Build history of the part. All positions in model axes, mm. A direction names the side the tool comes from. Coordinates: 2 decimals unless noted, no trailing zeros. Write each loop counter-clockwise with the first axis right and the second up, starting at its lowest first coordinate (ties: lowest second). Pieces come first, ordered by that corner, then holes.
from build123d import *

# Parameters (mm, degrees)
BASE_DISC_SKETCH_R           = 90
BASE_DISC_180_DEPTH          = 15
CLAMP_FRAME_WALL_DEPTH       = 70
TOP_JAW_PLATE_DEPTH          = 15
TABLE_RISER_SKETCH_R         = 60
TABLE_RISER_SKETCH_R_2       = 40
TABLE_RISER_DEPTH            = 40
RISER_START                  = -30
RISER_SLOTS_CUT_DEPTH        = 30
TABLE_PLATE_SKETCH_R         = 60
TABLE_PLATE_120_DEPTH        = 5
TABLE_BOLT_HOLES_SKETCH_R    = 5
TABLE_BOLT_HOLES_4X_10_DEPTH = 20
TABLE_RING_SKETCH_R          = 40
TABLE_RING_SKETCH_R_2        = 30
TABLE_RING_80_DEPTH          = 15
CENTRE_SPIGOT_SKETCH_R       = 20
CENTRE_SPIGOT_40_DEPTH       = 25


with BuildPart() as part:
    # Base Disc Sketch → Base Disc _180 (new body)
    with BuildSketch(Plane(origin=(0, 0, 0), x_dir=(1, 0, 0), z_dir=(0, 1, 0))):
        with Locations(Location((0, 0, 0), (0, 0, 270))):
            Circle(BASE_DISC_SKETCH_R)
    extrude(amount=BASE_DISC_180_DEPTH)

    # Clamp Frame Wall Sketch → Clamp Frame Wall (add)
    with BuildSketch(Plane(origin=(0, 15, 0), x_dir=(1, 0, 0), z_dir=(0, 1, 0))):
        with BuildLine():
            Line((0, -90), (0, -75))
            ThreePointArc((0, -75), (-75, 0), (0, 75))
            Line((0, 75), (0, 90))
            ThreePointArc((0, 90), (-90, 0), (0, -90))
        make_face()
    extrude(amount=CLAMP_FRAME_WALL_DEPTH)

    # Top Jaw Sketch → Top Jaw Plate (add)
    with BuildSketch(Plane(origin=(0, 85, 0), x_dir=(1, 0, 0), z_dir=(0, 1, 0))):
        with BuildLine():
            Line((0, 75), (0, 90))
            ThreePointArc((0, 90), (-90, 0), (0, -90))
            Line((0, -90), (0, -75))
            ThreePointArc((0, -75), (-75, 0), (0, 75))
        make_face()
        with BuildLine():
            Line((0, -75), (0, 75))
            ThreePointArc((0, 75), (-75, 0), (0, -75))
        make_face()
        with BuildLine():
            Line((83.180526567, 75), (0, 75))
            Line((0, 75), (0, -75))
            Line((0, -75), (49.749371855, -75))
            Line((49.749371855, -75), (83.180526567, -75))
            ThreePointArc((83.180526567, -75), (112, 0), (83.180526567, 75))
        make_face()
    extrude(amount=TOP_JAW_PLATE_DEPTH)

    # Table Riser Sketch → Table Riser (add)
    with BuildSketch(Plane(origin=(0, 100, 0), x_dir=(1, 0, 0), z_dir=(0, 1, 0))):
        with Locations(Location((0, 0, 0), (0, 0, 270))):
            Circle(TABLE_RISER_SKETCH_R)
        with Locations(Location((0, 0, 0), (0, 0, 270))):
            Circle(TABLE_RISER_SKETCH_R_2, mode=Mode.SUBTRACT)
    extrude(amount=TABLE_RISER_DEPTH)

    # Riser Slots Sketch → Riser Slots Cut (cut)
    with BuildSketch(Plane(origin=(0, 130, 0), x_dir=(1, 0, 0), z_dir=(0, 1, 0)).offset(RISER_START)):
        with BuildLine():
            Line((59.160797831, 10), (38.729833462, 10))
            ThreePointArc((38.729833462, 10), (28.284271247, 28.284271247), (10, 38.729833462))
            Line((10, 38.729833462), (10, 59.160797831))
            ThreePointArc((10, 59.160797831), (42.426406871, 42.426406871), (59.160797831, 10))
        make_face()
        with BuildLine():
            Line((-10, 59.160797831), (-10, 38.729833462))
            ThreePointArc((-10, 38.729833462), (-28.284271247, 28.284271247), (-38.729833462, 10))
            Line((-38.729833462, 10), (-59.160797831, 10))
            ThreePointArc((-59.160797831, 10), (-42.426406871, 42.426406871), (-10, 59.160797831))
        make_face()
        with BuildLine():
            Line((59.160797831, -10), (38.729833462, -10))
            ThreePointArc((38.729833462, -10), (28.284271247, -28.284271247), (10, -38.729833462))
            Line((10, -38.729833462), (10, -59.160797831))
            ThreePointArc((10, -59.160797831), (42.426406871, -42.426406871), (59.160797831, -10))
        make_face()
        with BuildLine():
            Line((-10, -59.160797831), (-10, -38.729833462))
            ThreePointArc((-10, -38.729833462), (-28.284271247, -28.284271247), (-38.729833462, -10))
            Line((-38.729833462, -10), (-59.160797831, -10))
            ThreePointArc((-59.160797831, -10), (-42.426406871, -42.426406871), (-10, -59.160797831))
        make_face()
    extrude(amount=RISER_SLOTS_CUT_DEPTH, mode=Mode.SUBTRACT)

    # Table Plate Sketch → Table Plate _120 (add)
    with BuildSketch(Plane(origin=(0, 140, 0), x_dir=(1, 0, 0), z_dir=(0, 1, 0))):
        with Locations(Location((0, 0, 0), (0, 0, 80.405931773))):
            Circle(TABLE_PLATE_SKETCH_R)
    extrude(amount=TABLE_PLATE_120_DEPTH)

    # Table Bolt Holes Sketch → Table Bolt Holes 4x_10 (cut)
    with BuildSketch(Plane(origin=(0, 145, 0), x_dir=(1, 0, 0), z_dir=(0, 1, 0))):
        with BuildLine():
            ThreePointArc((38.890872965, 38.890872965), (31.819805153, 38.890872965), (31.819805153, 31.819805153))
            Line((31.819805153, 31.819805153), (38.890872965, 38.890872965))
        make_face()
        with BuildLine():
            Line((38.890872965, 38.890872965), (31.819805153, 31.819805153))
            ThreePointArc((31.819805153, 31.819805153), (37.268756221, 30.735941397), (40.355339059, 35.355339059))
            ThreePointArc((40.355339059, 35.355339059), (39.974736722, 37.268756221), (38.890872965, 38.890872965))
        make_face()
        with Locations(Location((-35.355339059, 35.355339059, 0), (0, 0, 270))):
            Circle(TABLE_BOLT_HOLES_SKETCH_R)
        with Locations(Location((-35.355339059, -35.355339059, 0), (0, 0, 270))):
            Circle(TABLE_BOLT_HOLES_SKETCH_R)
        with Locations(Location((35.355339059, -35.355339059, 0), (0, 0, 270))):
            Circle(TABLE_BOLT_HOLES_SKETCH_R)
    extrude(amount=-TABLE_BOLT_HOLES_4X_10_DEPTH, mode=Mode.SUBTRACT)

    # Table Ring Sketch → Table Ring _80 (add)
    with BuildSketch(Plane(origin=(0, 145, 0), x_dir=(1, 0, 0), z_dir=(0, 1, 0))):
        with Locations(Location((0, 0, 0), (0, 0, 75.522487814))):
            Circle(TABLE_RING_SKETCH_R)
        with Locations(Location((0, 0, 0), (0, 0, 270))):
            Circle(TABLE_RING_SKETCH_R_2, mode=Mode.SUBTRACT)
    extrude(amount=TABLE_RING_80_DEPTH)

    # Centre Spigot Sketch → Centre Spigot _40 (add)
    with BuildSketch(Plane(origin=(0, 145, 0), x_dir=(1, 0, 0), z_dir=(0, 1, 0))):
        with Locations(Location((0, 0, 0), (0, 0, 270))):
            Circle(CENTRE_SPIGOT_SKETCH_R)
    extrude(amount=CENTRE_SPIGOT_40_DEPTH)


solid = part.part
(1) Slice it at A-A, the plane y = 157. List the corners of the cut face in (x, z), and give its area (3 significant figures).
(2) Flat gauge pins, fed straight in: P1, Ø22.5, axis at x = 45, y = 121.5, coming from the +Z side; P2, Ø7.5, axis at x = 34.5, y = 93, coming from the -Z side; P3, Ø14.5, axis at x = -32, z = 41.5, coming from the -Y side; P4, Ø10, axis at y = 122, z = 47, coming from the +X side. Where does each tip first touch, or does it go through?
(3) Slice it at D-D, the plane x = -64. List the corners of the cut face in (y, z), and give its area (3 significant figures).
(4) Two-plate mould, pull along X, no slides. Class faces 1 (the flat face through (0, 170, 0)), 2 (the cylindrical face through (1.32, 152.4, -29.97)), 3 (the flat face through (10, 115, -49)), 4 (the flat face through (-1, 140, 0)): pulls with the +X half, pulls with the -X half, needs draft (parallel to the pull), parting line crosses it, or undercut.
(5) 3-axis set-ups, long thin cutter, end or side, ignore diameter. For faces 5 (the flat face through (34, 130, 29)), 6 (the flat face through (17, 85, -1)), 7 (the flat face through (-27.4, 160, -13)): which of +Z, -Z, +X, -X, +Y, -Y reach the whole face in a straight line?
(6) Slice it at B-B, the plane x = 75. List the corners of the cut face in (y, z).
(7) Probe L1, parallel to Y at x = 33, z = -11; L2, parallel to Y at x = 65, z = 24; L3, parallel to Z at x = 0, y = 125. List the from-to ranges inside material, lowest first.
Results:
1. outline: circle Ø80 at (0, 0); circle Ø40 at (0, 0); hole circle Ø60 at (0, 0)
1. area: 3,460 mm2
2. P1: stops at z = 46.73
2. P2: stops at z = -75
2. P3: stops at y = 0
2. P4: stops at x = 10
3. outline: (0, -63.28) - (100, -63.28) - (100, 63.28) - (0, 63.28) - close; hole (15, -39.1) - (85, -39.1) - (85, 39.1) - (15, 39.1) - close
3. area: 7,180 mm2
4. face 1: needs draft
4. face 2: undercut
4. face 3: pulls with the +X half
4. face 4: undercut
5. face 5: +Z, +X
5. face 6: +X
5. face 7: +Y
6. outline: (0, -49.75) - (15, -49.75) - (15, 49.75) - (0, 49.75) - close; (85, -75) - (100, -75) - (100, 75) - (85, 75) - close
7. L1: y = 0 to 15, 85 to 100, 140 to 160
7. L2: y = 0 to 15, 85 to 100
7. L3: z = -60 to -40, 40 to 60
